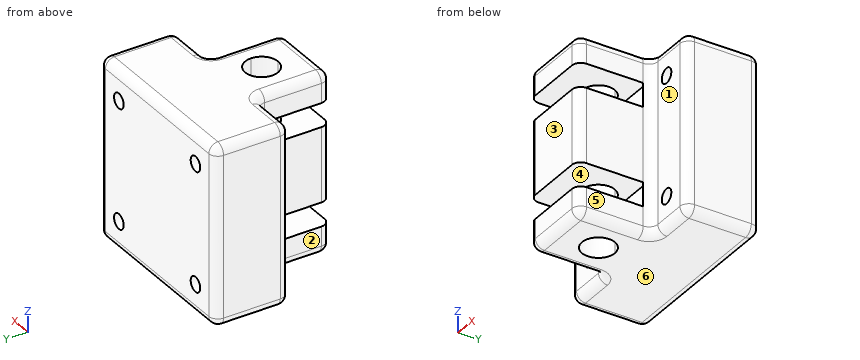
```python
from build123d import *

# Parameters (mm, degrees)
SKETCH1_W           = 17.5
SKETCH1_H           = 25
SKETCH1_W_2         = 12.5
BOSS_EXTRUDE1_DEPTH = 30
FILLET1_R           = 3
SKETCH2_W           = 25
SKETCH2_H           = 8
CUT_EXTRUDE1_DEPTH  = 23
SKETCH3_R           = 2.5
CUT_EXTRUDE2_DEPTH  = 50.244289009


with BuildPart() as part:
    # Sketch1 → Boss-Extrude1 (new, symmetric)
    with BuildSketch(Plane.XY):
        with BuildLine():
            Line((-12.5, 0), (0, 0))
            Line((0, 0), (0, 9.5))
            ThreePointArc((0, 9.5), (-5.5, 15), (0, 20.5))
            Line((0, 20.5), (0, 25))
            Line((0, 25), (-12.5, 25))
            Line((-12.5, 25), (-12.5, 0))
        make_face()
        with BuildLine():
            Line((0, 9.5), (0, 0))
            Line((0, 0), (12.5, 0))
            Line((12.5, 0), (12.5, 25))
            Line((12.5, 25), (0, 25))
            Line((0, 25), (0, 20.5))
            ThreePointArc((0, 20.5), (3.889087297, 18.889087297), (5.5, 15))
            ThreePointArc((5.5, 15), (3.889087297, 11.110912703), (0, 9.5))
        make_face()
        with Locations((21.25, 37.5)):
            Rectangle(SKETCH1_W, SKETCH1_H)
        with Locations((6.25, 37.5)):
            Rectangle(SKETCH1_W_2, SKETCH1_H)
        with Locations((-6.25, 37.5)):
            Rectangle(SKETCH1_W_2, SKETCH1_H)
        with Locations((-21.25, 37.5)):
            Rectangle(SKETCH1_W, SKETCH1_H)
    extrude(amount=BOSS_EXTRUDE1_DEPTH, both=True)

    # Fillet1
    fillet1_edges = [part.edges().sort_by_distance(p)[0] for p in [
        (0, 0, -30),
        (-12.5, 12.5, -30),
        (-21.25, 25, -30),
        (-30, 37.5, -30),
        (30, 37.5, 30),
        (0, 50, -30),
        (30, 37.5, -30),
        (21.25, 25, -30),
        (12.5, 12.5, -30),
        (0, 50, 30),
        (12.5, 0, 0),
        (-12.5, 0, 0),
        (-12.5, 25, 0),
        (-30, 25, 0),
        (-30, 50, 0),
        (30, 50, 0),
        (30, 25, 0),
        (12.5, 25, 0),
        (-30, 37.5, 30),
        (-21.25, 25, 30),
        (-12.5, 12.5, 30),
        (0, 0, 30),
        (12.5, 12.5, 30),
        (21.25, 25, 30),
    ]]
    fillet(fillet1_edges, radius=FILLET1_R)

    # Sketch2 → Cut-Extrude1 (cut)
    with BuildSketch(Plane.XZ):
        with Locations((0, 16.5)):
            Rectangle(SKETCH2_W, SKETCH2_H)
        with Locations((0, -16.5)):
            Rectangle(SKETCH2_W, SKETCH2_H)
    extrude(amount=-CUT_EXTRUDE1_DEPTH, mode=Mode.SUBTRACT)

    # Sketch3 → Cut-Extrude2 (cut, through all)
    with BuildSketch(Plane.XZ.offset(-25)):
        with Locations(Location((20, 20, 0), (0, 0, 270))):
            Circle(SKETCH3_R)
        with Locations(Location((20, -20, 0), (0, 0, 270))):
            Circle(SKETCH3_R)
        with Locations(Location((-20, -20, 0), (0, 0, 270))):
            Circle(SKETCH3_R)
        with Locations(Location((-20, 20, 0), (0, 0, 270))):
            Circle(SKETCH3_R)
    extrude(amount=-CUT_EXTRUDE2_DEPTH, mode=Mode.SUBTRACT)


solid = part.part
```
Geometry: final body of the model. Coordinates: model frame, mm. Face numbers are marked on the shaded views. A direction names the side the tool comes from. Round coordinates to 2 decimals unless told otherwise and drop trailing zeros. Write each loop counter-clockwise with the first axis right and the second up, starting at its lowest first coordinate (ties: lowest second). Pieces come first, ordered by that corner, then holes. Notation, with made-up numbers: (36.25, 65) -> (88.25, 65) arc R30 ccw to (88.25, 104) -> close; hole circle Ø8 at (21, -9.5). An arc over 180 degrees is marked (long way). Return JSON: item names as keys, results as strings.
Q1. Section C-C on y = 14. Return the cut outline in (x, z), and give its area (3 significant figures).
From the geometry:
{"outline": "(-12.5, -27) arc R3 ccw to (-9.5, -30) -> (-5.41, -30) -> (-5.41, -20.5) -> (-12.5, -20.5) -> close; (-12.5, -12.5) -> (-5.41, -12.5) -> (-5.41, 12.5) -> (-12.5, 12.5) -> close; (-12.5, 20.5) -> (-5.41, 20.5) -> (-5.41, 30) -> (-9.5, 30) arc R3 ccw to (-12.5, 27) -> close; (5.41, -30) -> (9.5, -30) arc R3 ccw to (12.5, -27) -> (12.5, -20.5) -> (5.41, -20.5) -> close; (5.41, -12.5) -> (12.5, -12.5) -> (12.5, 12.5) -> (5.41, 12.5) -> close; (5.41, 20.5) -> (12.5, 20.5) -> (12.5, 27) arc R3 ccw to (9.5, 30) -> (5.41, 30) -> close", "area": "616 mm2"}
Q2. Set-up query: the marked faces 1, 2 and 3. Return all of +Z, -Z, +X, -X, +Y, -Y with unobstructed straight access to the full face (end or side cutting, diameter ignored); none if empty.
From the geometry:
{"face 1": "+Z, -Z, +X, -Y", "face 2": "+Z, -Z, -X, -Y", "face 3": "+Z, -Z, +X, -X, -Y"}
Q3. Ray query, line 1 (X direction, y = 43, z = -20); line 2 (X direction, y = 34, z = 20.5); line 3 (Z direction, x = -19, y = 35.5). Return the intervals inside material, ascending.
From the geometry:
{"line 1": "-30 to -22.5, -17.5 to 17.5, 22.5 to 30", "line 2": "-30 to -22.45, -17.55 to 17.55, 22.45 to 30", "line 3": "-30 to -22.29, -17.71 to 17.71, 22.29 to 30"}
Q4. First-contact query: pin 1 Ø5.5 at (y, z) = (14, -2.5) entering from +X; pin 2 Ø0.8 at (y, z) = (22.5, -14.5) entering from +X; pin 3 Ø6 at (x, z) = (23, -8.5) entering from -Y. Flat tips, straight axial feed; report the tip coordinate or a pass-through.
From the geometry:
{"pin 1": "x = 12.5", "pin 2": "x = 12.64", "pin 3": "y = 25"}
Q5. Section B-B on x = 20. Return the cut outline in (y, z).
From the geometry:
{"outline": "(25, -27) arc R3 ccw to (28, -30) -> (47, -30) arc R3 ccw to (50, -27) -> (50, -22.5) -> (25, -22.5) -> close; (25, -17.5) -> (50, -17.5) -> (50, 17.5) -> (25, 17.5) -> close; (25, 22.5) -> (50, 22.5) -> (50, 27) arc R3 ccw to (47, 30) -> (28, 30) arc R3 ccw to (25, 27) -> close"}
Q6. Section A-A on y = 8. Return the cut outline in (x, z), and give its area (3 significant figures).
From the geometry:
{"outline": "(-12.5, -27) arc R3 ccw to (-9.5, -30) -> (9.5, -30) arc R3 ccw to (12.5, -27) -> (12.5, -20.5) -> (-12.5, -20.5) -> close; (-12.5, -12.5) -> (12.5, -12.5) -> (12.5, 12.5) -> (-12.5, 12.5) -> close; (-12.5, 20.5) -> (12.5, 20.5) -> (12.5, 27) arc R3 ccw to (9.5, 30) -> (-9.5, 30) arc R3 ccw to (-12.5, 27) -> close", "area": "1,090 mm2"}
Q7. Section D-D on y = 19. Return the cut outline in (x, z).
From the geometry:
{"outline": "(-12.5, -27) arc R3 ccw to (-9.5, -30) -> (-3.77, -30) -> (-3.77, -20.5) -> (-12.5, -20.5) -> close; (-12.5, -12.5) -> (-3.77, -12.5) -> (-3.77, 12.5) -> (-12.5, 12.5) -> close; (-12.5, 20.5) -> (-3.77, 20.5) -> (-3.77, 30) -> (-9.5, 30) arc R3 ccw to (-12.5, 27) -> close; (3.77, -30) -> (9.5, -30) arc R3 ccw to (12.5, -27) -> (12.5, -20.5) -> (3.77, -20.5) -> close; (3.77, -12.5) -> (12.5, -12.5) -> (12.5, 12.5) -> (3.77, 12.5) -> close; (3.77, 20.5) -> (12.5, 20.5) -> (12.5, 27) arc R3 ccw to (9.5, 30) -> (3.77, 30) -> close"}
Q8. Mould query, pull axis Z, two halves, no side actions, for the marked faces 4, 5 and 6. Classes: +Z half, -Z half, draft (parallel to the pull), parting line (faces both ways), or undercut.
From the geometry:
{"face 4": "undercut", "face 5": "draft", "face 6": "-Z half"}
